Could you check a few things on this model? Use its own coordinates, in mm. A direction names the side the tool comes from. Coordinates: 2 decimals unless noted, no trailing zeros. Loops run counter-clockwise (first coordinate to the right, second up) from the corner with the lowest first, then second, coordinate; pieces in that order, holes last. Notation, with made-up numbers: (50, -31) -> (71, -31) arc R10 cw to (71, -23) -> close; hole circle Ø8 at (75, -28). An arc over 180 degrees is marked (long way). One line per question, with ' | ' between items. Start each with the question number.
(1) Suppose I cut it at C-C (y = 5.5). Give the number of separate pieces and of enclosed holes in the cut face, plus the area to 3 significant figures.
(2) Suppose I cut it at A-A (z = -210). Please give me the cut outline in (x, y).
(3) I'm going to push flat-ended pins straight in: pin 1 Ø5 at (y, z) = (17.5, 417) entering from -X; pin 2 Ø2 at (x, y) = (187, 20.5) entering from +Z; pin 3 Ø1.5 at (x, y) = (-117.5, 25.5) entering from +Z. Where does each tip first touch, or does it pass through?
(4) Suppose I cut it at B-B (z = 105.5). Please give me the cut outline in (x, y).
(5) If I drill on line 1 along Z through (x, y) = (184, 18.5); line 2 along X through (y, z) = (24.75, 498); line 3 along Z through (x, y) = (-572.5, 18), over which ranges is the centre line in solid material (lowest first)?
(6) Which directions (+Z, -Z, +X, -X, +Y, -Y) give clear straight access to the entire face, cutting with the end or side of a thin tool? Please do faces 1 (the face through (724, 25, -124)), 2 (the face through (-645, 30, 213)).
```python
from build123d import *

# Parameters (mm, degrees)
SKETCH_1_R                = 810
EXTRUDE_1_DEPTH           = 25
SKETCH_2_R                = 730
EXTRUDE_2_DEPTH           = 5
CUT_EXTRUDE_1_REACH       = 1147.906
SKETCH_3_R                = 75
SKETCH_4_R                = 110
CUT_EXTRUDE_2_DEPTH       = 5
HOLE_WIZARD_M8_1_D        = 6.8
HOLE_WIZARD_25_5_25_5_1_D = 26
CUT_EXTRUDE_3_DEPTH       = 1146.905755287
CUT_EXTRUDE_3_DEPTH_BACK  = 1146.905755287
SKETCH_10_R               = 675


with BuildPart() as part:
    # 草图1 → 凸台-拉伸1 (new body)
    with BuildSketch(Plane(origin=(0, 0, 0), x_dir=(1, 0, 0), z_dir=(0, 1, 0))):
        with Locations(Location((0, 0, 0), (0, 0, 270))):
            Circle(SKETCH_1_R)
    extrude(amount=EXTRUDE_1_DEPTH)

    # 草图2 → 凸台-拉伸2 (add)
    with BuildSketch(Plane(origin=(0, 25, 0), x_dir=(1, 0, 0), z_dir=(0, 1, 0))):
        with Locations(Location((0, 0, 0), (0, 0, 270))):
            Circle(SKETCH_2_R)
    extrude(amount=EXTRUDE_2_DEPTH)

    # 草图3 → 切除-拉伸1 (cut, up to next)
    with BuildSketch(Plane(origin=(0, 30, 0), x_dir=(1, 0, 0), z_dir=(0, 1, 0)), mode=Mode.PRIVATE) as cut_extrude_1_sk1:
        with BuildLine():
            Line((130, 662.363193422), (130, -662.363193422))
            ThreePointArc((130, -662.363193422), (521.236510617, -428.879353665), (675, 0))
            ThreePointArc((675, 0), (521.236510617, 428.879353665), (130, 662.363193422))
        make_face()
    cut_extrude_1_tool1 = extrude(cut_extrude_1_sk1.sketch, amount=-CUT_EXTRUDE_1_REACH, mode=Mode.PRIVATE) & part.part
    # 草图3 → 切除-拉伸1 (cut, up to next)
    with BuildSketch(Plane(origin=(0, 30, 0), x_dir=(1, 0, 0), z_dir=(0, 1, 0)), mode=Mode.PRIVATE) as cut_extrude_1_sk2:
        with BuildLine():
            ThreePointArc((-130, 662.363193422), (-675, 0), (-130, -662.363193422))
            Line((-130, -662.363193422), (-130, 662.363193422))
        make_face()
    cut_extrude_1_tool2 = extrude(cut_extrude_1_sk2.sketch, amount=-CUT_EXTRUDE_1_REACH, mode=Mode.PRIVATE) & part.part
    # 草图3 → 切除-拉伸1 (cut, up to next)
    with BuildSketch(Plane(origin=(0, 30, 0), x_dir=(1, 0, 0), z_dir=(0, 1, 0)), mode=Mode.PRIVATE) as cut_extrude_1_sk3:
        with Locations(Location((0, 0, 0), (0, 0, 270))):
            Circle(SKETCH_3_R)
    cut_extrude_1_tool3 = extrude(cut_extrude_1_sk3.sketch, amount=-CUT_EXTRUDE_1_REACH, mode=Mode.PRIVATE) & part.part
    add(cut_extrude_1_tool1.solids().sort_by_distance((357.907844, 30, 0))[0], mode=Mode.SUBTRACT)
    add(cut_extrude_1_tool2.solids().sort_by_distance((-357.907844, 30, 0))[0], mode=Mode.SUBTRACT)
    add(cut_extrude_1_tool3.solids().sort_by_distance((0, 30, 0))[0], mode=Mode.SUBTRACT)

    # 草图4 → 切除-拉伸2 (cut)
    with BuildSketch(Plane(origin=(0, 30, 0), x_dir=(1, 0, 0), z_dir=(0, 1, 0))):
        with Locations(Location((0, 0, 0), (0, 0, 270))):
            Circle(SKETCH_4_R)
    extrude(amount=-CUT_EXTRUDE_2_DEPTH, mode=Mode.SUBTRACT)

    # M8 螺纹孔1 (through all)
    with Locations(Plane(origin=(0, 25, 0), x_dir=(1, 0, 0), z_dir=(0, 1, 0))):
        with Locations((0, 85), (85, 0), (0, -85), (-85, 0)):
            Hole(HOLE_WIZARD_M8_1_D / 2)

    # Ø25.5 (25.5) 直径孔1 (through all)
    with Locations(Plane(origin=(0, 25, 0), x_dir=(1, 0, 0), z_dir=(0, 1, 0))):
        with Locations((-59.354305918, 754.167962969), (59.354305918, 754.167962969), (176.601417757, 735.597844781), (289.500016584, 698.914866345), (395.270164208, 645.022284334), (491.307448562, 575.247112976), (575.247112976, 491.307448562), (645.022284334, 395.270164208), (698.914866345, 289.500016584), (735.597844781, 176.601417757), (754.167962969, 59.354305918), (754.167962969, -59.354305918), (735.597844781, -176.601417757), (698.914866345, -289.500016584), (645.022284334, -395.270164208), (575.247112976, -491.307448562), (491.307448562, -575.247112976), (395.270164208, -645.022284334), (289.500016584, -698.914866345), (176.601417757, -735.597844781), (59.354305918, -754.167962969), (-59.354305918, -754.167962969), (-176.601417757, -735.597844781), (-289.500016584, -698.914866345), (-395.270164208, -645.022284334), (-491.307448562, -575.247112976), (-575.247112976, -491.307448562), (-645.022284334, -395.270164208), (-698.914866345, -289.500016584), (-735.597844781, -176.601417757), (-754.167962969, -59.354305918), (-754.167962969, 59.354305918), (-735.597844781, 176.601417757), (-698.914866345, 289.500016584), (-645.022284334, 395.270164208), (-575.247112976, 491.307448562), (-491.307448562, 575.247112976), (-395.270164208, 645.022284334), (-289.500016584, 698.914866345), (-176.601417757, 735.597844781)):
            Hole(HOLE_WIZARD_25_5_25_5_1_D / 2)

    # 草图10 → 切除-拉伸3 (cut, two sides: drawn at the far end of the back side and taken through both)
    with BuildSketch(Plane(origin=(0, 30, 0), x_dir=(1, 0, 0), z_dir=(0, 1, 0)).offset(-CUT_EXTRUDE_3_DEPTH_BACK)):
        with Locations(Location((0, 0, 0), (0, 0, 270))):
            Circle(SKETCH_10_R)
    extrude(amount=CUT_EXTRUDE_3_DEPTH + CUT_EXTRUDE_3_DEPTH_BACK, mode=Mode.SUBTRACT)


solid = part.part
```
Checks:
1) separate pieces: 1 | enclosed holes: 41 | area: 609,000 mm^2
2) outline: (-782.3, 0) -> (-641.5, 0) -> (-641.5, 30) -> (-699.14, 30) -> (-699.14, 25) -> (-782.3, 25) -> close; (641.5, 0) -> (782.3, 0) -> (782.3, 25) -> (699.14, 25) -> (699.14, 30) -> (641.5, 30) -> close
3) pin 1: stops at x = -695.91 | pin 2: stops at z = 788.36 | pin 3: stops at z = 801.51
4) outline: (-803.1, 0) -> (-666.7, 0) -> (-666.7, 30) -> (-722.34, 30) -> (-722.34, 25) -> (-803.1, 25) -> close; (666.7, 0) -> (803.1, 0) -> (803.1, 25) -> (722.34, 25) -> (722.34, 30) -> (666.7, 30) -> close
5) line 1: z = -788.82 to -746.29, -724.91 to -649.44, 649.44 to 724.91, 746.29 to 788.82 | line 2: x = -638.82 to -586.39, -564.1 to -455.65, 455.65 to 564.1, 586.39 to 638.82 | line 3: z = -573.01 to -504.01, -478.6 to -357.59, 357.59 to 478.6, 504.01 to 573.01
6) face 1: +Y | face 2: +Z, -Z, +X, -X, +Y
